from build123d import *

# Parameters (mm, degrees)
LOBED_BASE_PLATE_DEPTH      = 20
SQUARE_POCKET_WALL_DEPTH    = 25
POCKET_HOLES_SKETCH_R       = 11.5
POCKET_FLOOR_HOLES_4X_DEPTH = 25
EDGE_FILLET_R12_A_R         = 12
EDGE_FILLET_R12_B_R         = 12
EDGE_FILLET_R12_C_R         = 12
EDGE_FILLET_R12_D_R         = 12
EDGE_FILLET_R12_E_R         = 12
EDGE_FILLET_R12_F_R         = 12
EDGE_FILLET_R12_G_R         = 12
EDGE_FILLET_R12_H_R         = 12
MOUNTING_HOLES_SKETCH_R     = 6.5
MOUNTING_HOLES_4X_DEPTH     = 25


with BuildPart() as part:
    # Lobed Base Profile → Lobed Base Plate (new body)
    with BuildSketch(Plane(origin=(0, 0, 0), x_dir=(1, 0, 0), z_dir=(0, 1, 0))):
        with BuildLine():
            Line((52.650346772, -81.259588286), (23.147950432, -76.577884476))
            ThreePointArc((23.147950432, -76.577884476), (0, -80), (-23.147950432, -76.577884476))
            Line((-23.147950432, -76.577884476), (-52.650346772, -81.259588286))
            ThreePointArc((-52.650346772, -81.259588286), (-74.246212025, -74.246212025), (-81.259588286, -52.650346772))
            Line((-81.259588286, -52.650346772), (-76.577884476, -23.147950432))
            ThreePointArc((-76.577884476, -23.147950432), (-80, 0), (-76.577884476, 23.147950432))
            Line((-76.577884476, 23.147950432), (-81.259588286, 52.650346772))
            ThreePointArc((-81.259588286, 52.650346772), (-74.246212025, 74.246212025), (-52.650346772, 81.259588286))
            Line((-52.650346772, 81.259588286), (-23.147950432, 76.577884476))
            ThreePointArc((-23.147950432, 76.577884476), (0, 80), (23.147950432, 76.577884476))
            Line((23.147950432, 76.577884476), (52.650346772, 81.259588286))
            ThreePointArc((52.650346772, 81.259588286), (74.246212025, 74.246212025), (81.259588286, 52.650346772))
            Line((81.259588286, 52.650346772), (76.577884476, 23.147950432))
            ThreePointArc((76.577884476, 23.147950432), (80, 0), (76.577884476, -23.147950432))
            Line((76.577884476, -23.147950432), (81.259588286, -52.650346772))
            ThreePointArc((81.259588286, -52.650346772), (74.246212025, -74.246212025), (52.650346772, -81.259588286))
        make_face()
    extrude(amount=LOBED_BASE_PLATE_DEPTH)

    # Square Wall Profile → Square Pocket Wall (add)
    with BuildSketch(Plane(origin=(0, 20, 0), x_dir=(1, 0, 0), z_dir=(0, 1, 0))):
        with BuildLine():
            Line((50, -1.641590962), (50, -35))
            ThreePointArc((50, -35), (45.606601718, -45.606601718), (35, -50))
            Line((35, -50), (-35, -50))
            ThreePointArc((-35, -50), (-45.606601718, -45.606601718), (-50, -35))
            Line((-50, -35), (-50, 35))
            ThreePointArc((-50, 35), (-45.606601718, 45.606601718), (-35, 50))
            Line((-35, 50), (35, 50))
            ThreePointArc((35, 50), (45.606601718, 45.606601718), (50, 35))
            Line((50, 35), (50, -1.641590962))
        make_face()
        with BuildLine():
            Line((44, -1.641590962), (44, -29))
            ThreePointArc((44, -29), (39.606601718, -39.606601718), (29, -44))
            Line((29, -44), (-29, -44))
            ThreePointArc((-29, -44), (-39.606601718, -39.606601718), (-44, -29))
            Line((-44, -29), (-44, 29))
            ThreePointArc((-44, 29), (-39.606601718, 39.606601718), (-29, 44))
            Line((-29, 44), (29, 44))
            ThreePointArc((29, 44), (39.606601718, 39.606601718), (44, 29))
            Line((44, 29), (44, -1.641590962))
        make_face(mode=Mode.SUBTRACT)
    extrude(amount=SQUARE_POCKET_WALL_DEPTH)

    # Pocket Holes Sketch → Pocket Floor Holes 4x (cut)
    with BuildSketch(Plane(origin=(0, 20, 0), x_dir=(1, 0, 0), z_dir=(0, 1, 0))):
        with Locations(Location((22, -22, 0), (0, 0, 270))):
            Circle(POCKET_HOLES_SKETCH_R)
        with Locations(Location((22, 22, 0), (0, 0, 270))):
            Circle(POCKET_HOLES_SKETCH_R)
        with Locations(Location((-22, 22, 0), (0, 0, 270))):
            Circle(POCKET_HOLES_SKETCH_R)
        with Locations(Location((-22, -22, 0), (0, 0, 270))):
            Circle(POCKET_HOLES_SKETCH_R)
    extrude(amount=-POCKET_FLOOR_HOLES_4X_DEPTH, mode=Mode.SUBTRACT)

    # Edge Fillet R12 A
    edge_fillet_r12_a_edges = [part.edges().sort_by_distance(p)[0] for p in [
        (23.147950432, 10, 76.577884476),
    ]]
    fillet(edge_fillet_r12_a_edges, radius=EDGE_FILLET_R12_A_R)

    # Edge Fillet R12 B
    edge_fillet_r12_b_edges = [part.edges().sort_by_distance(p)[0] for p in [
        (-23.147950432, 10, 76.577884476),
    ]]
    fillet(edge_fillet_r12_b_edges, radius=EDGE_FILLET_R12_B_R)

    # Edge Fillet R12 C
    edge_fillet_r12_c_edges = [part.edges().sort_by_distance(p)[0] for p in [
        (23.147950432, 10, -76.577884476),
    ]]
    fillet(edge_fillet_r12_c_edges, radius=EDGE_FILLET_R12_C_R)

    # Edge Fillet R12 D
    edge_fillet_r12_d_edges = [part.edges().sort_by_distance(p)[0] for p in [
        (-23.147950432, 10, -76.577884476),
    ]]
    fillet(edge_fillet_r12_d_edges, radius=EDGE_FILLET_R12_D_R)

    # Edge Fillet R12 E
    edge_fillet_r12_e_edges = [part.edges().sort_by_distance(p)[0] for p in [
        (76.577884476, 10, -23.147950432),
    ]]
    fillet(edge_fillet_r12_e_edges, radius=EDGE_FILLET_R12_E_R)

    # Edge Fillet R12 F
    edge_fillet_r12_f_edges = [part.edges().sort_by_distance(p)[0] for p in [
        (76.577884476, 10, 23.147950432),
    ]]
    fillet(edge_fillet_r12_f_edges, radius=EDGE_FILLET_R12_F_R)

    # Edge Fillet R12 G
    edge_fillet_r12_g_edges = [part.edges().sort_by_distance(p)[0] for p in [
        (-76.577884476, 10, 23.147950432),
    ]]
    fillet(edge_fillet_r12_g_edges, radius=EDGE_FILLET_R12_G_R)

    # Edge Fillet R12 H
    edge_fillet_r12_h_edges = [part.edges().sort_by_distance(p)[0] for p in [
        (-76.577884476, 10, -23.147950432),
    ]]
    fillet(edge_fillet_r12_h_edges, radius=EDGE_FILLET_R12_H_R)

    # Mounting Holes Sketch → Mounting Holes 4x (cut)
    with BuildSketch(Plane(origin=(0, 20, 0), x_dir=(1, 0, 0), z_dir=(0, 1, 0))):
        with Locations(Location((65, 65, 0), (0, 0, 270))):
            Circle(MOUNTING_HOLES_SKETCH_R)
        with Locations(Location((65, -65, 0), (0, 0, 270))):
            Circle(MOUNTING_HOLES_SKETCH_R)
        with Locations(Location((-65, -65, 0), (0, 0, 270))):
            Circle(MOUNTING_HOLES_SKETCH_R)
        with Locations(Location((-65, 65, 0), (0, 0, 270))):
            Circle(MOUNTING_HOLES_SKETCH_R)
    extrude(amount=-MOUNTING_HOLES_4X_DEPTH, mode=Mode.SUBTRACT)


solid = part.part
The model under review builds one solid part; all positions refer to its coordinate system, in mm. A direction names the side the tool comes from. Coordinates: 2 decimals unless noted, no trailing zeros. Write each loop counter-clockwise with the first axis right and the second up, starting at its lowest first coordinate (ties: lowest second). Pieces come first, ordered by that corner, then holes. Notation, with made-up numbers: (-3.5, -8) - (9.5, -8) arc R31 ccw to (9.5, 21) - close; hole circle Ø7 at (73.5, 24). An arc over 180 degrees is marked (long way). Answer as CSV lines item,"result".
(1) We need section D-D (x = -65). Give the boundary of the cut face in (y, z), plus the area to 3 significant figures.
Data:
outline,"(0, -80.1) - (20, -80.1) - (20, -71.5) - (0, -71.5) - close; (0, -58.5) - (20, -58.5) - (20, 58.5) - (0, 58.5) - close; (0, 71.5) - (20, 71.5) - (20, 80.1) - (0, 80.1) - close"
area,"2,680 mm2"
(2) For line 1 along X through (y, z) = (11.25, 22); line 2 along Z through (x, y) = (13.5, 40.5); line 3 along Z through (x, y) = (-66.5, 6), list the stretches that pass through material, from the lowest coordinate up. Write a range as [from, to].
Data:
line 1,"x = [-76.99, -33.5], [-10.5, 10.5], [33.5, 76.99]"
line 2,"z = [-50, -44], [44, 50]"
line 3,"z = [-79.51, -71.32], [-58.68, 58.68], [71.32, 79.51]"
(3) Clearance check with flat-ended pins moving along their axes: pin 1 Ø2 at (y, z) = (6, 14.5) entering from -X; pin 2 Ø12.5 at (y, z) = (32, -14) entering from +X; pin 3 Ø10 at (x, z) = (54.5, 44) entering from +Y. State where each tip first meets the part, or that it passes through.
Data:
pin 1,"stops at x = -78.85"
pin 2,"stops at x = 50"
pin 3,"stops at y = 20"
(4) Tool access review of faces 4 (the flat face through (79.097, 9.86, 39.02)), 5 (the cylindrical face through (39.72, 32.33, 39.49)), 6 (the flat face through (-39.02, 9.86, 79.097)), 7 (the flat face through (0, 32, -50)), 8 (the flat face through (-79.156, 9.86, 39.397)): name each direction out of +Z, -Z, +X, -X, +Y, -Y from which nothing blocks a thin tool from reaching the whole face with its end or side.
Data:
face 4,"+X, +Y, -Y"
face 5,"+Y"
face 6,"+Z, +Y, -Y"
face 7,"-Z, +X, -X, +Y"
face 8,"-X, +Y, -Y"
(5) Mouldability with a two-part tool opening along Z and no side actions: class faces 1 (the cylindrical face through (0, 10, 80)), 2 (the cylindrical face through (45.49, 32.33, -45.72)), 3 (the cylindrical face through (-39.49, 32.33, 39.72)) as pulls with the +Z half, pulls with the -Z half, needs draft (parallel to the pull), parting line crosses it, or undercut.
Data:
face 1,"pulls with the +Z half"
face 2,"pulls with the -Z half"
face 3,"undercut"
(6) We need section C-C (y = 4.5). Count the separate pieces of the cut face and the enclosed holes in it, plus the area to 3 significant figures.
Data:
separate pieces,"1"
enclosed holes,"8"
area,"22,800 mm2"
(7) We need section B-B (z = 13). Give the boundary of the cut face in (x, y), plus the area to 3 significant figures.
Data:
outline,"(-78.94, 0) - (-29.16, 0) - (-29.16, 20) - (-44, 20) - (-44, 45) - (-50, 45) - (-50, 20) - (-78.94, 20) - close; (-14.84, 0) - (14.84, 0) - (14.84, 20) - (-14.84, 20) - close; (29.16, 0) - (78.94, 0) - (78.94, 20) - (50, 20) - (50, 45) - (44, 45) - (44, 20) - (29.16, 20) - close"
area,"2,880 mm2"
(8) We need section A-A (y = 37.5). Give the boundary of the cut face in (x, z).
Data:
outline,"(-50, -35) arc R15 ccw to (-35, -50) - (35, -50) arc R15 ccw to (50, -35) - (50, 35) arc R15 ccw to (35, 50) - (-35, 50) arc R15 ccw to (-50, 35) - close; hole (-44, -29) arc R15 ccw to (-29, -44) - (29, -44) arc R15 ccw to (44, -29) - (44, 29) arc R15 ccw to (29, 44) - (-29, 44) arc R15 ccw to (-44, 29) - close"
